Can you work these out from the model? Positions are in its coordinate system, mm. Round coordinates to 2 decimals unless told otherwise and drop trailing zeros. Order: outer loops, then holes, each group sorted by start corner. A loop starts at its lowest first (then second) coordinate and runs counter-clockwise, first axis right, second up.
Q1. Will these pins go through, and if not, where does the flat tip stop? P1, Ø1.5, axis at x = 3, z = 3.5, coming from the +Y side; P2, Ø3, axis at y = -2.5, z = 1.5, coming from the -X side.
Q2. If I drill on line 1 (X direction, y = -9.25, z = 3.65); line 2 (Y direction, x = 8.5, z = 4.15); line 3 (X direction, y = -10.25, z = 2.4), over which ranges is the centre line in solid material (lowest first)?
Q3. If we section it at A-A (x = 8.75): Please give me the cut outline in (y, z).
Q4. If we section it at B-B (z = 3.2): Please give me the cut outline in (x, y).
Q5. If we section it at C-C (y = -7.25): Please give me the cut outline in (x, z), plus the area to 3 significant figures.
Q6. We'd pull the mould along Y, two halves only. Please class faces 1 (the face through (11.36, -7.6, 3.04)), 2 (the face through (1, -2, 3)), 3 (the face through (13.99, -14.15, 3.04)), 4 (the face through (8, -5, 0)): pulls with the +Y half, pulls with the -Y half, needs draft (parallel to the pull), parting line crosses it, or undercut.
Q7. If we section it at D-D (x = 15): Please give me the cut outline in (y, z), plus the area to 3 significant figures.
from build123d import *

# Parameters (mm, degrees)
SKETCH1_W           = 17
SKETCH1_H           = 17
BOSS_EXTRUDE1_DEPTH = 6
FILLET1_R           = 10
FILLET2_R           = 5
SKETCH2_R           = 3
CUT_EXTRUDE1_DEPTH  = 6


with BuildPart() as part:
    # Sketch1 → Boss-Extrude1 (new body)
    with BuildSketch(Plane.XY):
        with Locations((8.5, -8.5)):
            Rectangle(SKETCH1_W, SKETCH1_H)
    extrude(amount=BOSS_EXTRUDE1_DEPTH)

    # Fillet1
    fillet1_edges = [part.edges().sort_by_distance(p)[0] for p in [
        (17, -17, 3),
    ]]
    fillet(fillet1_edges, radius=FILLET1_R)

    # Fillet2
    fillet2_edges = [part.edges().sort_by_distance(p)[0] for p in [
        (0, 0, 3),
    ]]
    fillet(fillet2_edges, radius=FILLET2_R)

    # Sketch2 → Cut-Extrude1 (cut)
    with BuildSketch(Plane.XY.offset(6)):
        with Locations((8.5, -8.5)):
            Circle(SKETCH2_R)
    extrude(amount=-CUT_EXTRUDE1_DEPTH, mode=Mode.SUBTRACT)


solid = part.part
Solution:
1. P1: stops at y = -0.16
1. P2: stops at x = 0.1
2. line 1: x = 0 to 5.6, 11.4 to 16.74
2. line 2: y = -16.89 to -11.5, -5.5 to 0
2. line 3: x = 0 to 6.06, 10.94 to 16.46
3. outline: (-16.85, 0) - (-11.49, 0) - (-11.49, 6) - (-16.85, 6) - close; (-5.51, 0) - (0, 0) - (0, 6) - (-5.51, 6) - close
4. outline: (0, -17) - (7, -17) arc R10 ccw to (17, -7) - (17, 0) - (5, 0) arc R5 ccw to (0, -5) - close; hole circle Ø6 at (8.5, -8.5)
5. outline: (0, 0) - (5.77, 0) - (5.77, 6) - (0, 6) - close; (11.23, 0) - (17, 0) - (17, 6) - (11.23, 6) - close
5. area: 69.3 mm2
6. face 1: undercut
6. face 2: pulls with the +Y half
6. face 3: pulls with the -Y half
6. face 4: needs draft
7. outline: (-13, 0) - (0, 0) - (0, 6) - (-13, 6) - close
7. area: 78.0 mm2
